Read the model definition and answer for the solid it produces. Units are mm, in the model's axes. Coordinates: 2 decimals unless noted, no trailing zeros. Loops run counter-clockwise (first coordinate to the right, second up) from the corner with the lowest first, then second, coordinate; pieces in that order, holes last. Notation, with made-up numbers: M 16.25,-11 L 70.25,-11 A22 cw 70.25,20 Z; hole C 14.25,-33 d10. An arc over 180 degrees is marked long. Use one line per item in the form item = value. Start each with the question number.
1. Flat-ended cylindrical pins translate along their axes: pin 1 (12 mm diameter, centred on y = -35, z = 12.5, fed in from +X); pin 2 (1 mm diameter, centred on x = 125.5, y = -1, fed in from +Z); pin 3 (10 mm diameter, centred on x = -69, y = -6.5, fed in from -Z). Find the tip coordinate at first contact, or state that the pin passes through.
2. The part is cut by section A-A (y = 0). Give the vertices of the cut face in (x, z), plus the area to 3 significant figures.
3. For a pull along X with two mould halves and no side action, classify faces 1 (the flat face through (-2, 2, 49)), 2 (the flat face through (36, 2, 25)), 3 (the cylindrical face through (18.28, 28.67, 12.08)) as released by +X, released by -X, zero draft, split by the parting line, or undercut.
4. The part is cut by section D-D (z = 43). Give the vertices of the cut face in (x, y), plus the area to 3 significant figures.
5. Find the intervals of material crossed by probe 1 along X at (y, z) = (-2, 8); probe 2 along Z at (x, y) = (101.5, 1.5); probe 3 along Z at (x, y) = (-74, 138), in increasing order. Write a range as [from, to].
6. The part is cut by section C-C (z = 13.5). Give the vertices of the cut face in (x, y), plus the area to 3 significant figures.
from build123d import *

# Parameters (mm, degrees)
SKETCH1_R           = 34
BOSS_EXTRUDE1_DEPTH = 50
SKETCH2_R           = 175
BOSS_EXTRUDE2_DEPTH = 25
SKETCH3_R           = 150
CUT_EXTRUDE1_DEPTH  = 1
CUT_EXTRUDE1_DRAFT  = -45
FILLET1_R           = 0.5
CHAMFER1_SIZE       = 3


with BuildPart() as part:
    # Sketch1 → Boss-Extrude1 (new body)
    with BuildSketch(Plane.XY):
        Circle(SKETCH1_R)
    extrude(amount=BOSS_EXTRUDE1_DEPTH)

    # Sketch2 → Boss-Extrude2 (add)
    with BuildSketch(Plane.XY.offset(50)):
        Circle(SKETCH2_R)
    extrude(amount=-BOSS_EXTRUDE2_DEPTH)


with BuildPart() as cut_extrude1_tool:
    # Sketch3 → Cut-Extrude1 (with draft: the straight prism first)
    with BuildSketch(Plane.XY.offset(50)):
        Circle(SKETCH3_R)
    extrude(amount=-CUT_EXTRUDE1_DEPTH)
    # Cut-Extrude1: the draft: its side faces are tilted about the plane it starts from
    cut_extrude1_sides = [cut_extrude1_tool.faces().sort_by_distance(p)[0] for p in [
        (-150, 0, 49.5),
    ]]
    draft(cut_extrude1_sides, Plane.XY.offset(50), CUT_EXTRUDE1_DRAFT)


with BuildPart() as part_1:
    add(part.part)

    # Cut-Extrude1: cut by cut_extrude1_tool
    add(cut_extrude1_tool.part, mode=Mode.SUBTRACT)

    # Fillet1
    fillet1_edges = [part_1.edges().sort_by_distance(p)[0] for p in [
        (-34, 0, 25),
    ]]
    fillet(fillet1_edges, radius=FILLET1_R)

    # Chamfer1
    chamfer1_edges = [part_1.edges().sort_by_distance(p)[0] for p in [
        (-175, 0, 50),
    ]]
    chamfer(chamfer1_edges, length=CHAMFER1_SIZE)


solid = part_1.part
Computed values:
q1.pin_1 = 17.75
q1.pin_2 = 49
q1.pin_3 = 25
q2.outline = M -175,25 L -34.5,25 A0.5 cw -34,24.5 L -34,0 L 34,0 L 34,24.5 A0.5 cw 34.5,25 L 175,25 L 175,47 L 172,50 L 150,50 L 149,49 L -149,49 L -150,50 L -172,50 L -175,47 Z
q2.area = 10,100 mm²
q3.face_1 = undercut
q3.face_2 = zero draft
q3.face_3 = split by the parting line
q4.outline = C 0,0 d350
q4.area = 96,200 mm²
q5.probe_1 = [-33.94, 33.94]
q5.probe_2 = [25, 49]
q5.probe_3 = [25, 50]
q6.outline = C 0,0 d68
q6.area = 3,630 mm²
